For this review, take the finished solid that the model builds, in its own axes (mm). A direction names the side the tool comes from. Round coordinates to 2 decimals unless told otherwise and drop trailing zeros. Write each loop counter-clockwise with the first axis right and the second up, starting at its lowest first coordinate (ties: lowest second). Pieces come first, ordered by that corner, then holes. Notation, with made-up numbers: M 46,85.25 L 54,85.25 A15 cw 54,89.25 Z; hole C -37.75,-20 d1. An arc over 180 degrees is marked long. Answer in a Markdown table with one row per item.
```python
from build123d import *

# Parameters (mm, degrees)
SKETCH1_W           = 45
SKETCH1_H           = 151
BOSS_EXTRUDE1_DEPTH = 20
SKETCH2_W           = 39
SKETCH2_H           = 145
CUT_EXTRUDE1_DEPTH  = 82.280378936
SKETCH3_R           = 3.25
CUT_EXTRUDE2_DEPTH  = 88.299770905
CUT_EXTRUDE3_DEPTH  = 149.092032196
CHAMFER1_SIZE       = 3
FILLET1_R           = 2
FILLET2_R           = 8


with BuildPart() as part:
    # Sketch1 → Boss-Extrude1 (new body)
    with BuildSketch(Plane(origin=(0, 0, 0), x_dir=(1, 0, 0), z_dir=(0, 1, 0))):
        Rectangle(SKETCH1_W, SKETCH1_H)
    extrude(amount=BOSS_EXTRUDE1_DEPTH)

    # Sketch2 → Cut-Extrude1 (cut, through all)
    with BuildSketch(Plane(origin=(0, 20, 0), x_dir=(1, 0, 0), z_dir=(0, 1, 0))):
        with Locations((3, 3)):
            Rectangle(SKETCH2_W, SKETCH2_H)
    extrude(amount=-CUT_EXTRUDE1_DEPTH, mode=Mode.SUBTRACT)

    # Sketch3 → Cut-Extrude2 (cut, through all)
    with BuildSketch(Plane(origin=(-16.5, 0, 0), x_dir=(0, 0, -1), z_dir=(1, 0, 0))):
        with Locations((69.5, 10)):
            Circle(SKETCH3_R)
    extrude(amount=-CUT_EXTRUDE2_DEPTH, mode=Mode.SUBTRACT)

    # Sketch4 → Cut-Extrude3 (cut, through all)
    with BuildSketch(Plane(origin=(0, 0, 69.5), x_dir=(-1, 0, 0), z_dir=(0, 0, -1))):
        with BuildLine():
            Line((-12.5, 13.5), (7.5, 13.5))
            ThreePointArc((7.5, 13.5), (11, 10), (7.5, 6.5))
            Line((7.5, 6.5), (-12.5, 6.5))
            ThreePointArc((-12.5, 6.5), (-16, 10), (-12.5, 13.5))
        make_face()
    extrude(amount=-CUT_EXTRUDE3_DEPTH, mode=Mode.SUBTRACT)

    # Chamfer1
    chamfer1_edges = [part.edges().sort_by_distance(p)[0] for p in [
        (22.5, 20, 72.5),
        (-19.5, 0, -75.5),
        (-19.5, 20, -75.5),
        (22.5, 0, 72.5),
    ]]
    chamfer(chamfer1_edges, length=CHAMFER1_SIZE)

    # Fillet1
    fillet1_edges = [part.edges().sort_by_distance(p)[0] for p in [
        (-16.5, 10, 69.5),
    ]]
    fillet(fillet1_edges, radius=FILLET1_R)

    # Fillet2
    fillet2_edges = [part.edges().sort_by_distance(p)[0] for p in [
        (-22.5, 10, 75.5),
    ]]
    fillet(fillet2_edges, radius=FILLET2_R)


solid = part.part
```
Q1. Take a section at B-B (y = 10). State the section outline as (x, z) points.
Found:
| item | result |
|---|---|
| outline | M -22.5,-75.5 L -16.5,-75.5 L -16.5,-72.75 L -22.5,-72.75 Z; M -22.5,-66.25 L -16.5,-66.25 L -16.5,67.5 A2 cw -14.5,69.5 L -11,69.5 L -11,75.5 L -14.5,75.5 A8 ccw -22.5,67.5 Z; M 16,69.5 L 22.5,69.5 L 22.5,75.5 L 16,75.5 Z |
Q2. Take a section at D-D (x = -18). State the section outline as (y, z) points, then the cut area to 3 significant figures.
Found:
| item | result |
|---|---|
| outline | M 0,-72.5 L 3,-75.5 L 17,-75.5 L 20,-72.5 L 20,74.69 L 0,74.69 Z; hole C 10,-69.5 d6.5 |
| area | 2,960 mm² |
Q3. For probe 1 along Y at (x, z) = (-19.05, -69.5); probe 2 along X at (y, z) = (18.75, 38); probe 3 along Z at (x, y) = (-1.5, 17), list the stretches that pass through material, from the lowest coordinate up.
Found:
| item | result |
|---|---|
| probe 1 | 0 to 6.75, 13.25 to 20 |
| probe 2 | -22.5 to -16.5 |
| probe 3 | 69.5 to 75.5 |
Q4. Mouldability with a two-part tool opening along Y and no side actions: class faces 1 (the face through (-17, 20, 12)), 2 (the face through (3, 13.5, 72)), 3 (the face through (-11, 10, 72)), 4 (the face through (-22.5, 10, -3)) as +Y half, -Y half, draft (parallel to the pull), parting line (faces both ways), or undercut.
Found:
| item | result |
|---|---|
| face 1 | +Y half |
| face 2 | undercut |
| face 3 | undercut |
| face 4 | draft |
Q5. Take a section at A-A (z = -69.5). State the section outline as (x, y) points, then the cut area to 3 significant figures.
Found:
| item | result |
|---|---|
| outline | M -22.5,0 L -16.5,0 L -16.5,6.75 L -22.5,6.75 Z; M -22.5,13.25 L -16.5,13.25 L -16.5,20 L -22.5,20 Z |
| area | 81.0 mm² |
Q6. Take a section at C-C (x = 9). State the section outline as (y, z) points, then the cut area to 3 significant figures.
Found:
| item | result |
|---|---|
| outline | M 0,69.5 L 6.5,69.5 L 6.5,75.5 L 0,75.5 Z; M 13.5,69.5 L 20,69.5 L 20,75.5 L 13.5,75.5 Z |
| area | 78.0 mm² |
Q7. Insertion check: P1, Ø6, axis at y = 10, z = -69.5, coming from the -X side; P2, Ø6, axis at x = 8, y = 13, coming from the -Z side; P3, Ø6, axis at y = 14.5, z = -26.5, coming from the +X side. Each pin has a flat end and moves straight along its axis. Give the tip position at first contact, or say it passes through.
Found:
| item | result |
|---|---|
| P1 | through |
| P2 | z = 69.5 |
| P3 | x = -16.5 |
Q8. Machinability: for faces 5 (the face through (-17, 0, 12)), 6 (the face through (4, 15, 69.5)), 7 (the face through (16, 10, 72)), which of the approach directions +Z, -Z, +X, -X, +Y, -Y give a long, thin tool a straight path to every point of the face, cutting with its end or side? Answer none if there is none.
Found:
| item | result |
|---|---|
| face 5 | +Z, -Z, +X, -X, -Y |
| face 6 | -Z, +X, +Y, -Y |
| face 7 | +Z, -Z |
